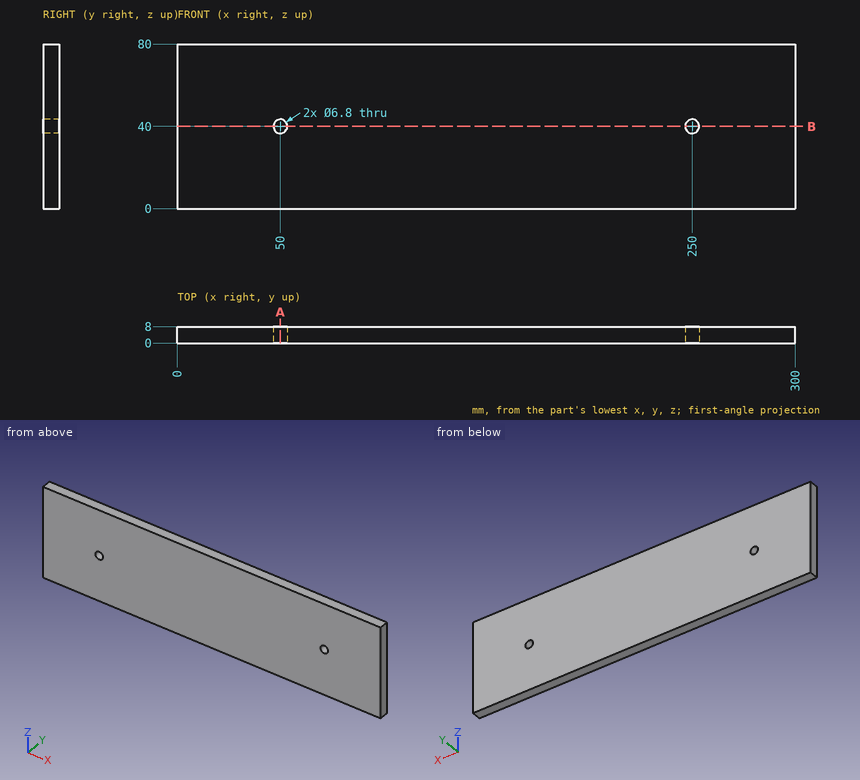
Part print with two shaded views. Sizes in mm from the minimum x, y, z corner. Give positions to 0.01 mm unless a question says otherwise; leave off trailing zeros. Order: outer loops, then holes, each group sorted by start corner. A loop starts at its lowest first (then second) coordinate and runs counter-clockwise, first axis right, second up.
1) Saw through at A-A, the plane x = 50. Write the cut outline in (y, z), then the cut area to 3 significant figures.
2) Saw through at B-B, the plane z = 40. Write the cut outline in (x, y).
3) Wall check: probe 1 along X at (y, z) = (3.75, 40); probe 2 along Z at (x, y) = (250, 3.5); probe 3 along X at (y, z) = (3, 41). Give the ranges that are in metal, low to high.
Computed:
1. outline: (0, 0) - (8, 0) - (8, 36.6) - (0, 36.6) - close; (0, 43.4) - (8, 43.4) - (8, 80) - (0, 80) - close
1. area: 586 mm2
2. outline: (0, 0) - (46.6, 0) - (46.6, 8) - (0, 8) - close; (53.4, 0) - (246.6, 0) - (246.6, 8) - (53.4, 8) - close; (253.4, 0) - (300, 0) - (300, 8) - (253.4, 8) - close
3. probe 1: x = 0 to 46.6, 53.4 to 246.6, 253.4 to 300
3. probe 2: z = 0 to 36.6, 43.4 to 80
3. probe 3: x = 0 to 46.75, 53.25 to 246.75, 253.25 to 300
